Part model, mm, in its own coordinate system. Face numbers are marked on the shaded views. A direction names the side the tool comes from. Round coordinates to 2 decimals unless told otherwise and drop trailing zeros. Write each loop counter-clockwise with the first axis right and the second up, starting at its lowest first coordinate (ties: lowest second). Pieces come first, ordered by that corner, then holes. Notation, with made-up numbers: M 44.5,17 L 81.5,17 A26 cw 81.5,39 Z; hole C 3.25,7.25 d3. An arc over 180 degrees is marked long. Use one line per item in the form item = value. Start each with the question number.
Item 1: Cut at C-C, the plane x = 35. Give the cut face in (y, z).
Item 2: Which spindle directions (+Z, -Z, +X, -X, +Y, -Y) get a long thin tool onto all of the face, cutting with end or side? Do the marked faces 1, 2 and 3. Say none if no direction does.
Item 3: Cut at D-D, the plane y = -48.5. Give the cut face in (x, z), then the cut area to 3 significant figures.
Item 4: Probe L1, parallel to Y at x = 35, z = 6; L2, parallel to Y at x = 35, z = 15; L3, parallel to X at y = -21.5, z = 1.75. List the from-to ranges inside material, lowest first.
Item 5: Flat gauge pins, fed straight in: pin 1 Ø1 at (x, y) = (36, -23.5) entering from -Z; pin 2 Ø10.5 at (x, y) = (35, -55) entering from +Z. Where does each tip first touch, or does it go through?
Item 6: Cut at B-B, the plane y = -10. Give the cut face in (x, z), then the cut area to 3 significant figures.
Item 7: Mould opens along X. For the marked faces 4, 5 and 6 say: +X half, -X half, draft (parallel to the pull), parting line (faces both ways), or undercut.
Item 8: Cut at A-A, the plane z = 9.75. Give the cut face in (x, y).
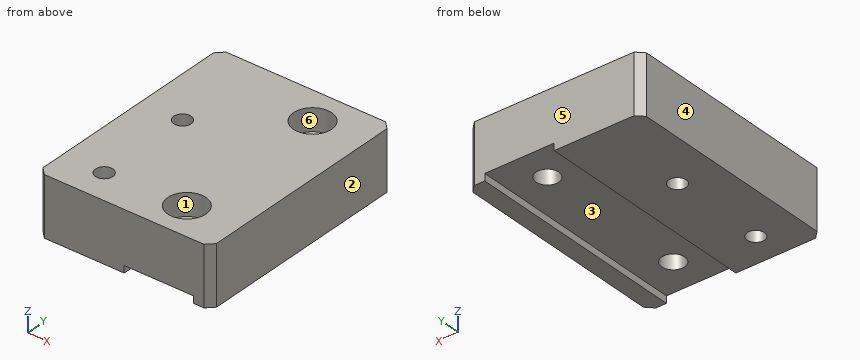
from build123d import *

# Parameters (mm, degrees)
SKETCH_2_W                     = 50
SKETCH_2_H                     = 65
EXTRUDE_1_DEPTH                = 17
SKETCH_3_W                     = 20
SKETCH_3_H                     = 2
CUT_EXTRUDE_1_DEPTH            = 84.749626865
CHAMFER_1_SIZE                 = 2
HOLE_WIZARD_M6_1_D             = 5
HOLE_WIZARD_M6_1_DEPTH         = 17
HOLE_WIZARD_M6_1_TIP           = 1.502151548
HOLE_WIZARD_M6_1_2_D           = 6.6
HOLE_WIZARD_M6_1_2_DEPTH       = 17
HOLE_WIZARD_M6_1_2_CBORE_D     = 11
HOLE_WIZARD_M6_1_2_CBORE_DEPTH = 6.4
HOLE_WIZARD_M6_1_2_TIP         = 1.982840043


with BuildPart() as part:
    # 草图2 → 凸台-拉伸1 (new body)
    with BuildSketch(Plane.XY):
        with Locations((25, -32.5)):
            Rectangle(SKETCH_2_W, SKETCH_2_H)
    extrude(amount=EXTRUDE_1_DEPTH)

    # 草图3 → 切除-拉伸1 (cut, through all)
    with BuildSketch(Plane.XZ.offset(65)):
        with Locations((35, 1)):
            Rectangle(SKETCH_3_W, SKETCH_3_H)
    extrude(amount=-CUT_EXTRUDE_1_DEPTH, mode=Mode.SUBTRACT)

    # 倒角1
    chamfer_1_edges = [part.edges().sort_by_distance(p)[0] for p in [
        (0, 0, 8.5),
        (50, 0, 8.5),
        (50, -65, 8.5),
        (0, -65, 8.5),
    ]]
    chamfer(chamfer_1_edges, length=CHAMFER_1_SIZE)

    # Hole Wizard M6 _1
    with Locations(Plane.XY.offset(17)):
        with Locations((12, -28), (12, -56)):
            Hole(HOLE_WIZARD_M6_1_D / 2, depth=HOLE_WIZARD_M6_1_DEPTH)
            with Locations((0, 0, -(HOLE_WIZARD_M6_1_DEPTH + HOLE_WIZARD_M6_1_TIP / 2))):  # 118° drill point
                Cone(0, HOLE_WIZARD_M6_1_D / 2, HOLE_WIZARD_M6_1_TIP, mode=Mode.SUBTRACT)

    # Hole Wizard M6 _1 2
    with Locations(Plane.XY.offset(17)):
        with Locations((35, -10), (35, -55)):
            CounterBoreHole(HOLE_WIZARD_M6_1_2_D / 2, HOLE_WIZARD_M6_1_2_CBORE_D / 2, HOLE_WIZARD_M6_1_2_CBORE_DEPTH, depth=HOLE_WIZARD_M6_1_2_DEPTH)
            with Locations((0, 0, -(HOLE_WIZARD_M6_1_2_DEPTH + HOLE_WIZARD_M6_1_2_TIP / 2))):  # 118° drill point
                Cone(0, HOLE_WIZARD_M6_1_2_D / 2, HOLE_WIZARD_M6_1_2_TIP, mode=Mode.SUBTRACT)


solid = part.part
Model answer:
q1.outline = M -65,2 L -58.3,2 L -58.3,10.6 L -60.5,10.6 L -60.5,17 L -65,17 Z; M -51.7,2 L -13.3,2 L -13.3,10.6 L -15.5,10.6 L -15.5,17 L -49.5,17 L -49.5,10.6 L -51.7,10.6 Z; M -6.7,2 L 0,2 L 0,17 L -4.5,17 L -4.5,10.6 L -6.7,10.6 Z
q2.face_1 = +Z
q2.face_2 = +Z, -Z, +X, +Y, -Y
q2.face_3 = -Z, +Y, -Y
q3.outline = M 0,0 L 25,0 L 25,2 L 45,2 L 45,0 L 50,0 L 50,17 L 0,17 Z
q3.area = 810 mm²
q4.L1 = -65 to -58.3, -51.7 to -13.3, -6.7 to 0
q4.L2 = -65 to -60.5, -49.5 to -15.5, -4.5 to 0
q4.L3 = 0 to 25, 45 to 50
q5.pin_1 = 2
q5.pin_2 = 10.6
q6.outline = M 0,0 L 25,0 L 25,2 L 31.7,2 L 31.7,10.6 L 29.5,10.6 L 29.5,17 L 0,17 Z; M 38.3,2 L 45,2 L 45,0 L 50,0 L 50,17 L 40.5,17 L 40.5,10.6 L 38.3,10.6 Z
q6.area = 683 mm²
q7.face_4 = -X half
q7.face_5 = draft
q7.face_6 = undercut
q8.outline = M 0,-63 L 2,-65 L 48,-65 L 50,-63 L 50,-2 L 48,0 L 2,0 L 0,-2 Z; hole C 12,-56 d5; hole C 12,-28 d5; hole C 35,-55 d6.6; hole C 35,-10 d6.6
